from build123d import *

# Parameters (mm, degrees)
SKETCH_1_R                = 3
EXTRUDE_1_DEPTH           = 25
CHAMFER_1_SIZE            = 3
SKETCH_2_R                = 1.072137289
CUT_EXTRUDE_1_DEPTH       = 50
HOLE_WIZARD_1_D           = 6.3
HOLE_WIZARD_1_CSINK_D     = 12
HOLE_WIZARD_1_CSINK_ANGLE = 90
SKETCH_4_W                = 23.881095176
SKETCH_4_H                = 12.5
SKETCH_4_W_2              = 26.910691004
CUT_EXTRUDE_2_DEPTH       = 50


with BuildPart() as part:
    # 草图1 → 拉伸1 (new, symmetric)
    with BuildSketch(Plane.XY):
        with BuildLine():
            Line((-7, 1), (0, 1))
            Line((0, 1), (0, 0))
            Line((0, 0), (18, 0))
            Line((18, 0), (18, 6))
            Line((18, 6), (-1.083920217, 6))
            Line((-1.083920217, 6), (-1.083920217, 8.748346358))
            Line((-1.083920217, 8.748346358), (-4, 11.5))
            Line((-4, 11.5), (-10, 11.5))
            Line((-10, 11.5), (-12.739624118, 8.748346358))
            ThreePointArc((-12.739624118, 8.748346358), (-11.821310929, 3.428591185), (-7, 1))
        make_face()
        with Locations((-7, 7)):
            Circle(SKETCH_1_R, mode=Mode.SUBTRACT)
    extrude(amount=EXTRUDE_1_DEPTH, both=True)

    # 倒角1
    chamfer_1_edges = [part.edges().sort_by_distance(p)[0] for p in [
        (18, 6, 0),
    ]]
    chamfer(chamfer_1_edges, length=CHAMFER_1_SIZE)

    # 草图2 → 切除-拉伸1 (cut)
    with BuildSketch(Plane(origin=(0, 6, 0), x_dir=(1, 0, 0), z_dir=(0, 1, 0))):
        with Locations(Location((8, 15, 0), (0, 0, 180))):
            Circle(SKETCH_2_R)
        with Locations(Location((8, -15, 0), (0, 0, 270))):
            Circle(SKETCH_2_R)
    extrude(amount=-CUT_EXTRUDE_1_DEPTH, mode=Mode.SUBTRACT)

    # 打孔尺寸开槽半沉头螺钉的类型1 (through all)
    with Locations(Plane(origin=(8, 6, -15), x_dir=(1, 0, 0), z_dir=(0, 1, 0))):
        with Locations((0, 0), (0, -30)):
            CounterSinkHole(HOLE_WIZARD_1_D / 2, HOLE_WIZARD_1_CSINK_D / 2, counter_sink_angle=HOLE_WIZARD_1_CSINK_ANGLE)

    # 草图4 → 切除-拉伸2 (cut)
    with BuildSketch(Plane(origin=(0, 11.5, 0), x_dir=(1, 0, 0), z_dir=(0, 1, 0))):
        with Locations((-11.940547588, 6.25)):
            Rectangle(SKETCH_4_W, SKETCH_4_H)
        with Locations((-13.455345502, -18.75)):
            Rectangle(SKETCH_4_W_2, SKETCH_4_H)
    extrude(amount=-CUT_EXTRUDE_2_DEPTH, mode=Mode.SUBTRACT)


solid = part.part
CAD build for the part. Positions are in the model's coordinates, mm. A direction names the side the tool comes from. Give positions to 0.01 mm unless a question says otherwise; leave off trailing zeros. Loops run counter-clockwise (first coordinate to the right, second up) from the corner with the lowest first, then second, coordinate; pieces in that order, holes last. Notation, with made-up numbers: M 40,-32 L 76,-32 A28 ccw 76,-4 Z; hole C 15,36.25 d1. An arc over 180 degrees is marked long. Write each question's results on one line, items separated by ' | '.
Q1. Band-saw the part on B-B on x = -0.5. Write the cut outline in (y, z), and give its area (3 significant figures).
Geometry check:
outline: M 1,-25 L 6,-25 L 6,-12.5 L 1,-12.5 Z; M 1,0 L 6,0 L 6,12.5 L 1,12.5 Z | area: 125 mm²
Q2. Probe probe 1 along Z at (x, y) = (8, 1.85); probe 2 along Z at (x, y) = (9.5, 1.25); probe 3 along Y at (x, z) = (-7, -19). List the from-to ranges inside material, lowest first.
Geometry check:
probe 1: z = -25 to -18.15, -11.85 to 11.85, 18.15 to 25 | probe 2: z = -25 to -17.77, -12.23 to 12.23, 17.77 to 25 | probe 3: y = 1 to 4, 10 to 11.5
Q3. Band-saw the part on D-D on z = 15. Write the cut outline in (x, y).
Geometry check:
outline: M 0,0 L 4.85,0 L 4.85,3.15 L 2,6 L 0,6 Z; M 11.15,0 L 18,0 L 18,3 L 15,6 L 14,6 L 11.15,3.15 Z
Q4. Flat gauge pins, fed straight in: P1, Ø5, axis at y = 3.5, z = 3, coming from the -X side; P2, Ø1, axis at y = 3, z = 17, coming from the -X side; P3, Ø4, axis at y = 1.5, z = 4.5, coming from the -X side; P4, Ø8, axis at x = 13.5, z = 16, coming from the -Y side. Where does each tip first touch, or does it go through?
Geometry check:
P1: stops at x = -12.92 | P2: stops at x = 0 | P3: stops at x = -11.87 | P4: stops at y = 0
Q5. Mould opens along Y. For faces 1 (the face through (-4.14, 7.9, -18.84)), 2 (the face through (-11.868, 3.492, 6.338)), 3 (the face through (-7, 11.5, 6)) say: pulls with the +Y half, pulls with the -Y half, needs draft (parallel to the pull), parting line crosses it, or undercut.
Geometry check:
face 1: undercut | face 2: parting line crosses it | face 3: pulls with the +Y half
Q6. Which spindle directions (+Z, -Z, +X, -X, +Y, -Y) get a long thin tool onto all of the face, cutting with end or side? Do faces 4 (the face through (-4, 1, -19)), 5 (the face through (-5, 4, 12.5)), 6 (the face through (7, 6, 0)), 7 (the face through (-5, 4, -12.5)). Say none if no direction does.
Geometry check:
face 4: +Z, -Z, -X, -Y | face 5: +Z, -X, +Y, -Y | face 6: +Z, -Z, +X, +Y | face 7: -X, +Y, -Y
Q7. Band-saw the part on C-C on y = 7. Write the cut outline in (x, z), and give its area (3 significant figures).
Geometry check:
outline: M -13,-25 L -10,-25 L -10,-12.5 L -13,-12.5 Z; M -13,0 L -10,0 L -10,12.5 L -13,12.5 Z; M -4,-25 L -1.08,-25 L -1.08,-12.5 L -4,-12.5 Z; M -4,0 L -1.08,0 L -1.08,12.5 L -4,12.5 Z | area: 148 mm²
Q8. Band-saw the part on A-A on z = -15. Write the cut outline in (x, y), and give its area (3 significant figures).
Geometry check:
outline: M -12.74,8.75 A6 ccw -7,1 L 0,1 L 0,0 L 4.85,0 L 4.85,3.15 L 2,6 L -1.08,6 L -1.08,8.75 L -4,11.5 L -10,11.5 Z; M 11.15,0 L 18,0 L 18,3 L 15,6 L 14,6 L 11.15,3.15 Z; hole C -7,7 d6 | area: 143 mm²
